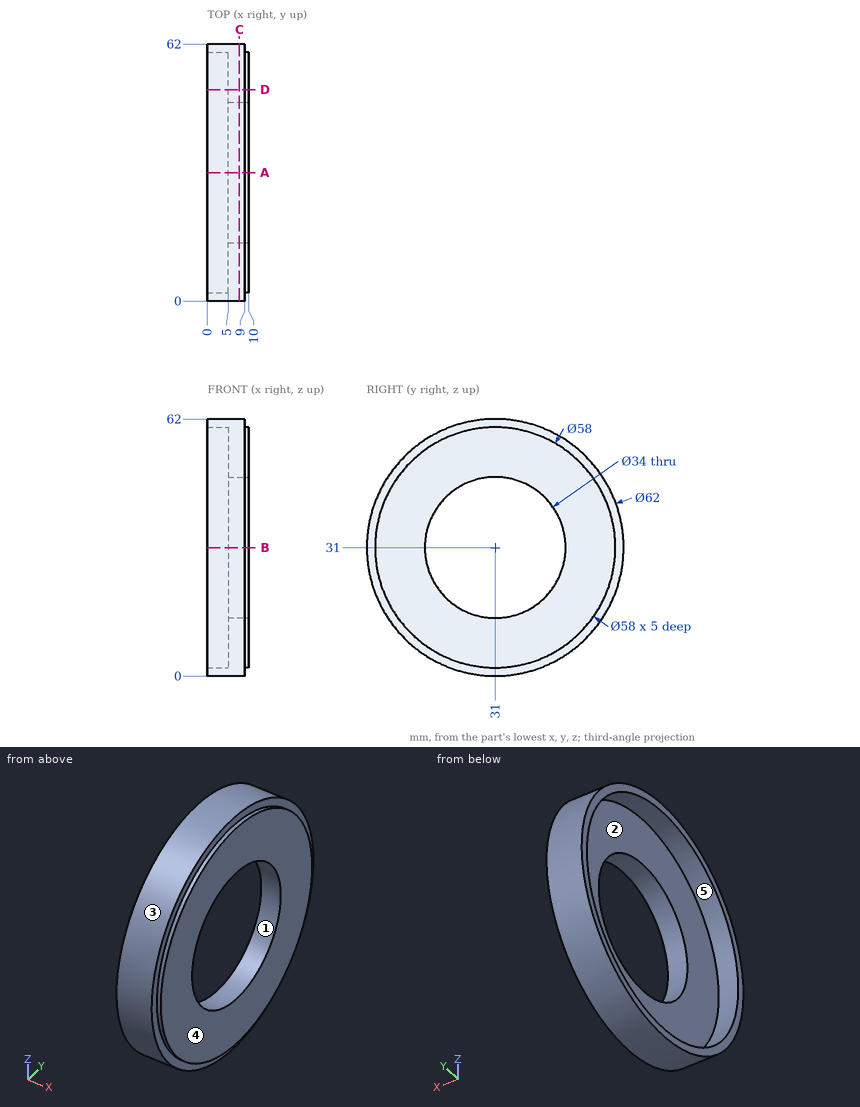
Could you check a few things on this drawing? It's one solid part, dimensions in mm from its lowest x, y, z. A direction names the side the tool comes from. Coordinates: 2 decimals unless noted, no trailing zeros. Write each loop counter-clockwise with the first axis right and the second up, starting at its lowest first coordinate (ties: lowest second). Pieces come first, ordered by that corner, then holes.
1) If I drill on line 1 (Y direction, x = 8.1, z = 31); line 2 (Y direction, x = 1.4, z = 31); line 3 (X direction, y = 13, z = 28.5), over which ranges is the centre line in solid material (lowest first)?
Filled in:
line 1: y = 0 to 14, 48 to 62
line 2: y = 0 to 2, 60 to 62
line 3: x = 5 to 10
2) Thinking about a two-plate mould opening in Y: for the marked faces 3, 4 and 5, which applies, +Y half, -Y half, draft (parallel to the pull), parting line (faces both ways), or undercut?
Filled in:
face 3: parting line
face 4: draft
face 5: undercut
3) If we section it at D-D (y = 51): List the corners of the cut face in (x, z) for me, plus the area to 3 significant figures.
Filled in:
outline: (0, 7.31) - (9, 7.31) - (9, 10) - (10, 10) - (10, 52) - (9, 52) - (9, 54.69) - (0, 54.69) - (0, 52) - (5, 52) - (5, 10) - (0, 10) - close
area: 258 mm2
4) Which directions (+Z, -Z, +X, -X, +Y, -Y) give clear straight access to the entire face, cutting with the end or side of a thin tool? Please do the marked faces 1 and 2.
Filled in:
face 1: +X, -X
face 2: -X
5) I'm going to push flat-ended pins straight in: pin 1 (3 mm diameter, centred on x = 5.5, y = 44.5, fed in from -Z); pin 2 (1 mm diameter, centred on x = 2, y = 50.5, fed in from -Z); pin 3 (5 mm diameter, centred on x = 1.5, z = 21, fed in from -Y). Where does each tip first touch, or does it pass through?
Filled in:
pin 1: stops at z = 2.42
pin 2: stops at z = 6.51
pin 3: stops at y = 0.92
6) If we section it at C-C (x = 7.75): List the corners of the cut face in (y, z) for me.
Filled in:
outline: circle Ø62 at (31, 31); hole circle Ø34 at (31, 31)
7) If we section it at A-A (y = 31): List the corners of the cut face in (x, z) for me.
Filled in:
outline: (0, 0) - (9, 0) - (9, 2) - (10, 2) - (10, 14) - (5, 14) - (5, 2) - (0, 2) - close; (0, 60) - (5, 60) - (5, 48) - (10, 48) - (10, 60) - (9, 60) - (9, 62) - (0, 62) - close
